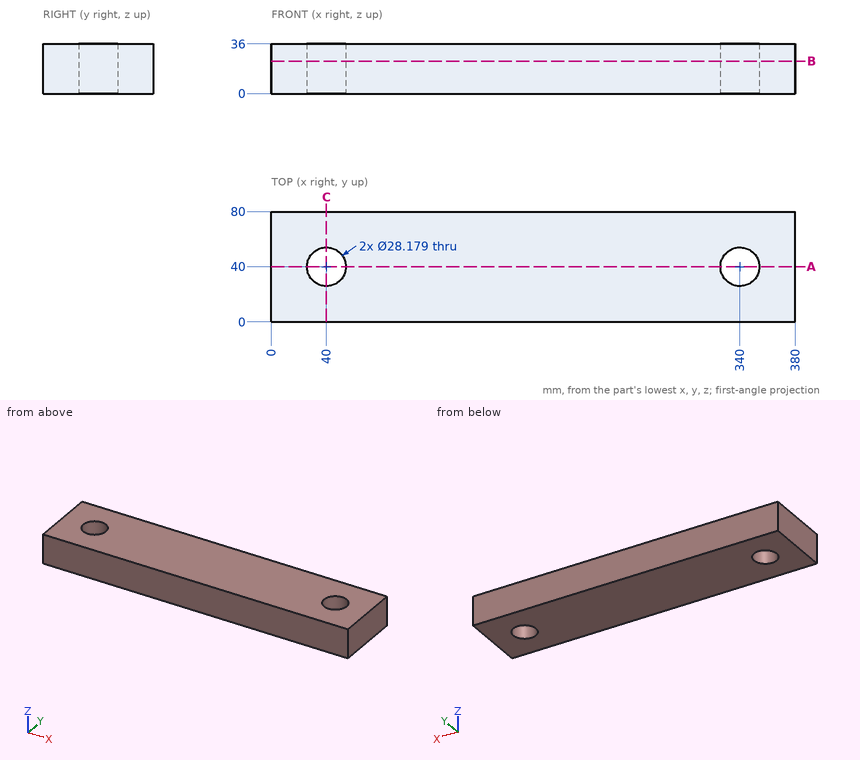
Answer from the drawing. Dimensions are ordinates in mm from the lowest x, y and z of the part. Coordinates: 2 decimals unless noted, no trailing zeros. Write each loop counter-clockwise with the first axis right and the second up, starting at its lowest first coordinate (ties: lowest second). Pieces come first, ordered by that corner, then holes. Notation, with made-up numbers: (-2.75, 88.25) - (13.25, 88.25) arc R25 cw to (13.25, 122.25) - close; hole circle Ø2 at (18.25, 35.25). An arc over 180 degrees is marked (long way). Return JSON: item names as keys, results as strings.
1. The part is cut by section B-B on z = 23.5. Determine the outline of the cut face in (x, y), then the cut area to 3 significant figures.
Final values:
{"outline": "(0, 0) - (380, 0) - (380, 80) - (0, 80) - close; hole circle Ø28.18 at (40, 40); hole circle Ø28.18 at (340, 40)", "area": "29,200 mm^2"}
2. Consider line 1 along X through (y, z) = (39, 12); line 2 along X through (y, z) = (30.5, 30.5) (1 decimal); line 3 along Y through (x, z) = (340, 27.5). Determine where each line is inside the solid, lowest interval first.
Final values:
{"line 1": "0 to 25.95, 54.05 to 325.95, 354.05 to 380", "line 2": "0 to 29.6, 50.4 to 329.6, 350.4 to 380", "line 3": "0 to 25.91, 54.09 to 80"}
3. This flat-tipped pin is pushed along its axis until it touches: pin 1 Ø1 at (y, z) = (64.5, 16.5) entering from -X. Where does it stop, or does it pass through?
Final values:
{"pin 1": "x = 0"}
4. The part is cut by section A-A on y = 40. Determine the outline of the cut face in (x, z).
Final values:
{"outline": "(0, 0) - (25.91, 0) - (25.91, 36) - (0, 36) - close; (54.09, 0) - (325.91, 0) - (325.91, 36) - (54.09, 36) - close; (354.09, 0) - (380, 0) - (380, 36) - (354.09, 36) - close"}
5. The part is cut by section C-C on x = 40. Determine the outline of the cut face in (y, z), then the cut area to 3 significant figures.
Final values:
{"outline": "(0, 0) - (25.91, 0) - (25.91, 36) - (0, 36) - close; (54.09, 0) - (80, 0) - (80, 36) - (54.09, 36) - close", "area": "1,870 mm^2"}
